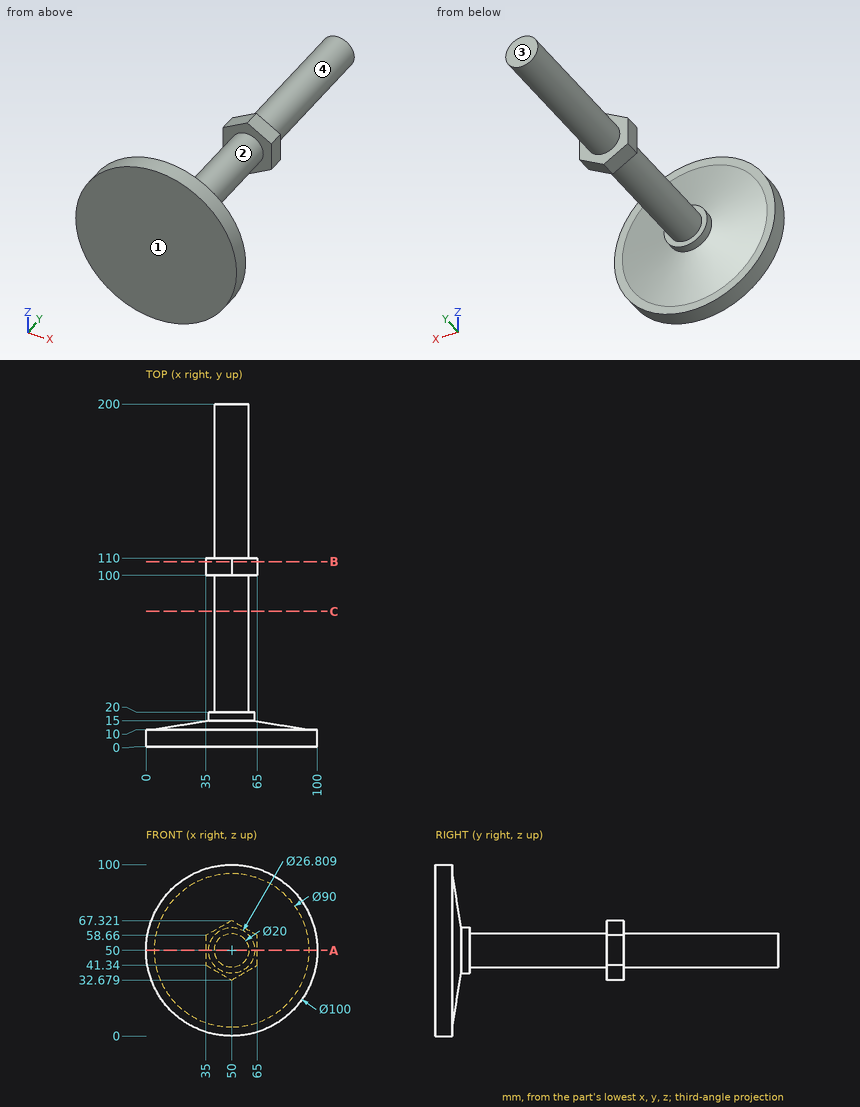
Here's the drawing with two shaded views (mm, measured from the low corner). I have some questions. Give positions to 0.01 mm unless a question says otherwise; leave off trailing zeros. Order: outer loops, then holes, each group sorted by start corner. A loop starts at its lowest first (then second) coordinate and runs counter-clockwise, first axis right, second up. Notation, with made-up numbers: M 3,86 L 27,86 A13 ccw 27,99 Z; hole C -30.5,25.5 d2. An arc over 180 degrees is marked long. Answer as a JSON object with one key per item and string values. Group by question number.
1) I'm going to push flat-ended pins straight in: pin 1 Ø3 at (y, z) = (103, 46.5) entering from +X; pin 2 Ø8 at (y, z) = (105, 48.5) entering from -X. Where does each tip first touch, or does it pass through?
2) Please list where these lines run through material, in increasing order: L1, parallel to Y at x = 52.5, z = 4.5; L2, parallel to Y at x = 66, z = 40.5; L3, parallel to Z at x = 50.5, y = 141. Write a range as [from, to].
3) Suppose I cut it at A-A, the plane z = 50. Write out the boundary of the cut face in (x, y) (1 decimal).
4) Suppose I cut it at B-B, the plane y = 108. Write out the boundary of the cut face in (x, z).
5) We'd pull the mould along Y, two halves only. Please class the marked faces 1, 2, 3 and 4: pulls with the +Y half, pulls with the -Y half, needs draft (parallel to the pull), parting line crosses it, or undercut.
6) Suppose I cut it at C-C, the plane y = 79. Write out the boundary of the cut face in (x, z), plus the area to 3 significant figures.
Results found:
{
 "1": {"pin 1": "x = 65", "pin 2": "x = 35"},
 "2": {"L1": "[0, 10]", "L2": "[0, 14.18]", "L3": "[40.01, 59.99]"},
 "3": {"outline": "M 0,0 L 100,0 L 100,10 L 95,10 L 63.4,15 L 63.4,20 L 60,20 L 60,100 L 65,100 L 65,110 L 60,110 L 60,200 L 40,200 L 40,110 L 35,110 L 35,100 L 40,100 L 40,20 L 36.6,20 L 36.6,15 L 5,10 L 0,10 Z"},
 "4": {"outline": "M 35,41.34 L 50,32.68 L 65,41.34 L 65,58.66 L 50,67.32 L 35,58.66 Z"},
 "5": {"face 1": "pulls with the -Y half", "face 2": "undercut", "face 3": "pulls with the +Y half", "face 4": "needs draft"},
 "6": {"outline": "C 50,50 d20", "area": "314 mm²"}
}
